```python
from build123d import *

# Parameters (mm, degrees)
SKETCH1_W                                           = 20
SKETCH1_H                                           = 400
BOSS_EXTRUDE1_DEPTH                                 = 12
HOLE_SIZE_BY_HEX_SOCKET_FLAT_COUNTERSUN_D           = 9
HOLE_SIZE_BY_HEX_SOCKET_FLAT_COUNTERSUN_CSINK_D     = 17.6
HOLE_SIZE_BY_HEX_SOCKET_FLAT_COUNTERSUN_CSINK_ANGLE = 90


with BuildPart() as part:
    # Sketch1 → Boss-Extrude1 (new body)
    with BuildSketch(Plane.XY):
        with Locations((10, 200)):
            Rectangle(SKETCH1_W, SKETCH1_H)
    extrude(amount=BOSS_EXTRUDE1_DEPTH)

    # Hole size (by hex socket flat countersunk head screw type)1 (through all)
    with Locations(Plane.XY.offset(12)):
        with Locations((10, 380), (10, 200), (10, 20)):
            CounterSinkHole(HOLE_SIZE_BY_HEX_SOCKET_FLAT_COUNTERSUN_D / 2, HOLE_SIZE_BY_HEX_SOCKET_FLAT_COUNTERSUN_CSINK_D / 2, counter_sink_angle=HOLE_SIZE_BY_HEX_SOCKET_FLAT_COUNTERSUN_CSINK_ANGLE)


solid = part.part
```
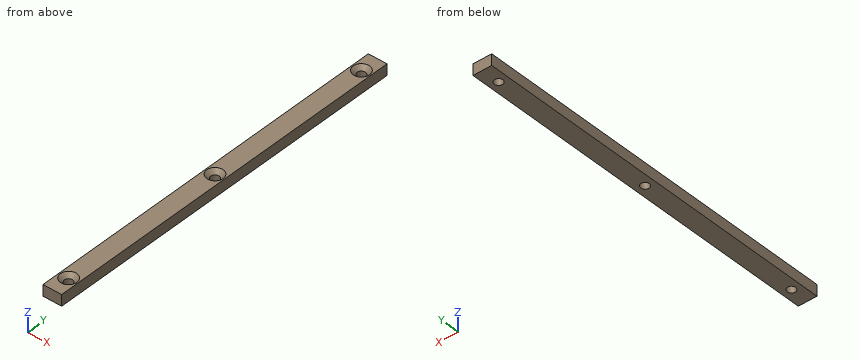
CAD build for the part. Positions are in the model's coordinates, mm. Round coordinates to 2 decimals unless told otherwise and drop trailing zeros. Order: outer loops, then holes, each group sorted by start corner. A loop starts at its lowest first (then second) coordinate and runs counter-clockwise, first axis right, second up. Notation, with made-up numbers: (85.5, -33.75) - (127.5, -33.75) arc R17 ccw to (127.5, -19.75) - close; hole circle Ø6 at (-5.75, -3). An arc over 180 degrees is marked (long way). Answer as CSV lines item,"result". Start each with the question number.
1. Drill centre lines: L1, parallel to Y at x = 10, z = 2; L2, parallel to X at y = 200, z = 1.75; L3, parallel to Y at x = 10.5, z = 10.75. Where is each one in solid material? Low to high. Write a range as [from, to].
2. Saw through at A-A, the plane y = 20. Write the cut outline in (x, z).
3. Pin check, flat tips, straight feed: pin 1 (2 mm diameter, centred on x = 9, y = 65.5, fed in from -Z); pin 2 (7 mm diameter, centred on x = 10, y = 20, fed in from -Z). Stop position of each tip, or through.
4. Saw through at C-C, the plane x = 10. Write the cut outline in (y, z).
5. Saw through at B-B, the plane z = 9.75. Write the cut outline in (x, y).
Model answer:
1,L1,"y = [0, 15.5], [24.5, 195.5], [204.5, 375.5], [384.5, 400]"
1,L2,"x = [0, 5.5], [14.5, 20]"
1,L3,"y = [0, 12.47], [27.53, 192.47], [207.53, 372.47], [387.53, 400]"
2,outline,"(0, 0) - (5.5, 0) - (5.5, 7.7) - (1.2, 12) - (0, 12) - close; (14.5, 0) - (20, 0) - (20, 12) - (18.8, 12) - (14.5, 7.7) - close"
3,pin 1,"stops at z = 0"
3,pin 2,"passes through"
4,outline,"(0, 0) - (15.5, 0) - (15.5, 7.7) - (11.2, 12) - (0, 12) - close; (24.5, 0) - (195.5, 0) - (195.5, 7.7) - (191.2, 12) - (28.8, 12) - (24.5, 7.7) - close; (204.5, 0) - (375.5, 0) - (375.5, 7.7) - (371.2, 12) - (208.8, 12) - (204.5, 7.7) - close; (384.5, 0) - (400, 0) - (400, 12) - (388.8, 12) - (384.5, 7.7) - close"
5,outline,"(0, 0) - (20, 0) - (20, 400) - (0, 400) - close; hole circle Ø13.1 at (10, 20); hole circle Ø13.1 at (10, 200); hole circle Ø13.1 at (10, 380)"
